```python
from build123d import *

# Parameters (mm, degrees)
EXTRUDE_1_DEPTH = 70
FILLET_1_R      = 5


with BuildPart() as part:
    # 草图1 → 凸台-拉伸1 (new body)
    with BuildSketch(Plane.XY):
        Polygon((0, 0), (100, 0), (100, -15), (75, -40), (50, -40), (25, -40), (0, -15), align=None)
    extrude(amount=EXTRUDE_1_DEPTH)

    # 圆角1
    fillet_1_edges = [part.edges().sort_by_distance(p)[0] for p in [
        (50, -40, 70),
        (100, -15, 35),
        (75, -40, 35),
        (25, -40, 35),
        (0, -15, 35),
        (87.5, -27.5, 70),
        (12.5, -27.5, 70),
        (87.5, -27.5, 0),
        (50, -40, 0),
        (12.5, -27.5, 0),
    ]]
    fillet(fillet_1_edges, radius=FILLET_1_R)


solid = part.part
```
Model file for the job. Use its own axes, mm. Coordinates: 2 decimals unless noted, no trailing zeros. Loops run counter-clockwise (first coordinate to the right, second up) from the corner with the lowest first, then second, coordinate; pieces in that order, holes last. Notation, with made-up numbers: M 38.5,-36 L 97.5,-36 A31 cw 97.5,2 Z; hole C 21.5,67.25 d8. An arc over 180 degrees is marked long. Use CSV: the item, a comma, the result in double quotes. Start each with the question number.
1. Flat gauge pin, fed straight in: pin 1 (1.5 mm diameter, centred on x = 75.5, z = 28, fed in from -Y). Where does the tip first touch, or does it go through?
2. Band-saw the part on A-A, the plane z = 38. List the corners of the cut face in (x, y), then the cut area to 3 significant figures.
3. Probe probe 1 along Y at (x, z) = (83, 39.5); probe 2 along Y at (x, z) = (5, 34); probe 3 along X at (y, z) = (-25, 4.5). List the from-to ranges inside material, lowest first. Write a range as [from, to].
Entries:
1,pin 1,"stops at y = -39.66"
2,outline,"M 0,-12.93 A5 ccw 1.46,-16.46 L 23.54,-38.54 A5 ccw 27.07,-40 L 72.93,-40 A5 ccw 76.46,-38.54 L 98.54,-16.46 A5 ccw 100,-12.93 L 100,0 L 0,0 Z"
2,area,"3,370 mm2"
3,probe 1,"y = [-32, 0]"
3,probe 2,"y = [-20, 0]"
3,probe 3,"x = [10.04, 89.96]"
